The model under review builds one solid part; all positions refer to its coordinate system, in mm. Face numbers are marked on the shaded views. A direction names the side the tool comes from. Coordinates: 2 decimals unless noted, no trailing zeros. Write each loop counter-clockwise with the first axis right and the second up, starting at its lowest first coordinate (ties: lowest second). Pieces come first, ordered by that corner, then holes. Notation, with made-up numbers: M 85.25,-9.5 L 100.25,-9.5 A29 ccw 100.25,12.5 Z; hole C -9.5,85.5 d9. An arc over 180 degrees is marked long. Answer as a JSON object with one key per item and string values.
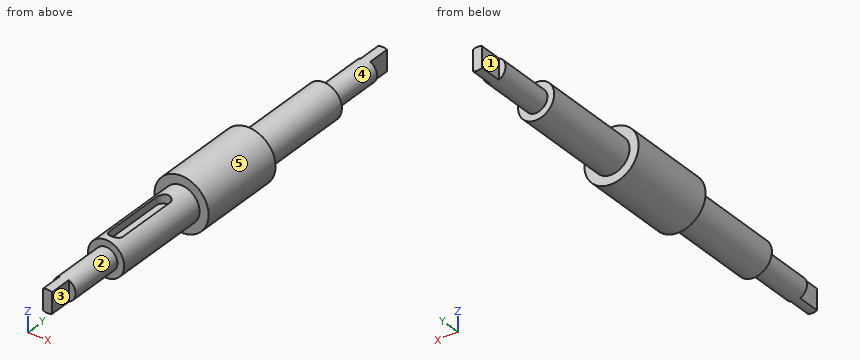
```python
from build123d import *

# Parameters (mm, degrees)
SKETCH1_R           = 6
BOSS_EXTRUDE1_DEPTH = 10
SKETCH2_R           = 4
BOSS_EXTRUDE2_DEPTH = 22.5
SKETCH3_R           = 2.5
BOSS_EXTRUDE3_DEPTH = 12.5
BOSS_EXTRUDE4_START = 22.5
SKETCH4_R           = 4
BOSS_EXTRUDE4_DEPTH = 22.5
BOSS_EXTRUDE5_START = 12.5
SKETCH5_R           = 2.5
BOSS_EXTRUDE5_DEPTH = 12.5
BOSS_EXTRUDE6_START = 5
BOSS_EXTRUDE6_DEPTH = 5
BOSS_EXTRUDE7_DEPTH = 5
CUT_EXTRUDE1_DEPTH  = 2


with BuildPart() as part:
    # Sketch1 → Boss-Extrude1 (new, symmetric)
    with BuildSketch(Plane(origin=(0, 0, 0), x_dir=(1, 0, 0), z_dir=(0, 1, 0))):
        with Locations(Location((0, 0, 0), (0, 0, 270))):
            Circle(SKETCH1_R)
    extrude(amount=BOSS_EXTRUDE1_DEPTH, both=True)

    # Sketch2 → Boss-Extrude2 (add)
    with BuildSketch(Plane(origin=(0, 10, 0), x_dir=(1, 0, 0), z_dir=(0, 1, 0))):
        with Locations(Location((0, 0, 0), (0, 0, 90))):
            Circle(SKETCH2_R)
    extrude(amount=BOSS_EXTRUDE2_DEPTH)

    # Sketch3 → Boss-Extrude3 (add)
    with BuildSketch(Plane(origin=(0, 32.5, 0), x_dir=(1, 0, 0), z_dir=(0, 1, 0))):
        with Locations(Location((0, 0, 0), (0, 0, 270))):
            Circle(SKETCH3_R)
    extrude(amount=BOSS_EXTRUDE3_DEPTH)

    # Sketch4 → Boss-Extrude4 (add)
    with BuildSketch(Plane.XZ.offset(10).offset(BOSS_EXTRUDE4_START)):
        with Locations(Location((0, 0, 0), (0, 0, 270))):
            Circle(SKETCH4_R)
    extrude(amount=-BOSS_EXTRUDE4_DEPTH)

    # Sketch5 → Boss-Extrude5 (add)
    with BuildSketch(Plane.XZ.offset(32.5).offset(BOSS_EXTRUDE5_START)):
        with Locations(Location((0, 0, 0), (0, 0, 90))):
            Circle(SKETCH5_R)
    extrude(amount=-BOSS_EXTRUDE5_DEPTH)

    # Sketch6 → Boss-Extrude6 (add)
    with BuildSketch(Plane(origin=(0, -45, 0), x_dir=(-1, 0, 0), z_dir=(0, -1, 0)).offset(BOSS_EXTRUDE6_START)):
        with BuildLine():
            Line((1, -2.291287847), (1, 2.291287847))
            ThreePointArc((1, 2.291287847), (0, 2.5), (-1, 2.291287847))
            Line((-1, 2.291287847), (-1, -2.291287847))
            ThreePointArc((-1, -2.291287847), (0, -2.5), (1, -2.291287847))
        make_face()
    extrude(amount=-BOSS_EXTRUDE6_DEPTH)

    # Sketch7 → Boss-Extrude7 (add)
    with BuildSketch(Plane(origin=(0, 45, 0), x_dir=(1, 0, 0), z_dir=(0, 1, 0))):
        with BuildLine():
            Line((-1, 2.291287847), (-1, -2.291287847))
            ThreePointArc((-1, -2.291287847), (0, -2.5), (1, -2.291287847))
            Line((1, -2.291287847), (1, 2.291287847))
            ThreePointArc((1, 2.291287847), (0, 2.5), (-1, 2.291287847))
        make_face()
    extrude(amount=BOSS_EXTRUDE7_DEPTH)

    # Sketch8 → Cut-Extrude1 (cut)
    with BuildSketch(Plane.XY.offset(4)):
        with BuildLine():
            Line((-1.5, -29.5), (-1.5, -15.5))
            ThreePointArc((-1.5, -15.5), (0, -14), (1.5, -15.5))
            Line((1.5, -15.5), (1.5, -29.5))
            ThreePointArc((1.5, -29.5), (0, -31), (-1.5, -29.5))
        make_face()
    extrude(amount=-CUT_EXTRUDE1_DEPTH, mode=Mode.SUBTRACT)


solid = part.part
```
(1) Add section C-C on y = 8. Give the boundary of the cut face in (x, z), and give its area (3 significant figures).
Results list:
{"outline": "C 0,0 d12", "area": "113 mm²"}
(2) For the marked faces 1, 2, 3, 4 and 5, list the 3-axis set-ups (+Z, -Z, +X, -X, +Y, -Y) from which the entire face can be reached by the end or side of a thin tool; tool diameter is ignored.
Results list:
{"face 1": "+Z, -Z, -X, +Y", "face 2": "-Y", "face 3": "+Z, -Z, +X, -Y", "face 4": "+Y", "face 5": "+Y, -Y"}
(3) For pin 1 Ø0.9 at (y, z) = (-22, 3) entering from +X; pin 2 Ø1.4 at (y, z) = (48, -1) entering from -X; pin 3 Ø4 at (x, y) = (-0.5, 34) entering from +Z, all flat-tipped, find the tip position at first contact; note any pin that passes through.
Results list:
{"pin 1": "x = 3.08", "pin 2": "x = -1", "pin 3": "z = 4"}
(4) Wall thickness on line 1 along Y through (x, z) = (-1.75, -3.25); line 2 along Y through (x, z) = (3.75, -2); line 3 along X through (y, z) = (45.5, -1.25): over which ranges is each line inside the solid? List them lowest first. Write a range as from..to.
Results list:
{"line 1": "-32.5..32.5", "line 2": "-10..10", "line 3": "-1..1"}
(5) Add section B-B on y = -34.5. Give the boundary of the cut face in (x, z).
Results list:
{"outline": "C 0,0 d5"}
(6) Add section A-A on z = 0. Give the boundary of the cut face in (x, y), and give its area (3 significant figures).
Results list:
{"outline": "M -6,-10 L -4,-10 L -4,-32.5 L -2.5,-32.5 L -2.5,-45 L -1,-45 L -1,-50 L 1,-50 L 1,-45 L 2.5,-45 L 2.5,-32.5 L 4,-32.5 L 4,-10 L 6,-10 L 6,10 L 4,10 L 4,32.5 L 2.5,32.5 L 2.5,45 L 1,45 L 1,50 L -1,50 L -1,45 L -2.5,45 L -2.5,32.5 L -4,32.5 L -4,10 L -6,10 Z", "area": "745 mm²"}
